Build history of the part. All positions in model axes, mm. Face numbers are marked on the shaded views. A direction names the side the tool comes from. Round coordinates to 2 decimals unless told otherwise and drop trailing zeros. Write each loop counter-clockwise with the first axis right and the second up, starting at its lowest first coordinate (ties: lowest second). Pieces come first, ordered by that corner, then holes. Notation, with made-up numbers: (-9.75, 77) -> (45.25, 77) arc R16 cw to (45.25, 92) -> close; hole circle Ø6 at (70.5, 57.5). An arc over 180 degrees is marked (long way). Return JSON: item names as keys, results as strings.
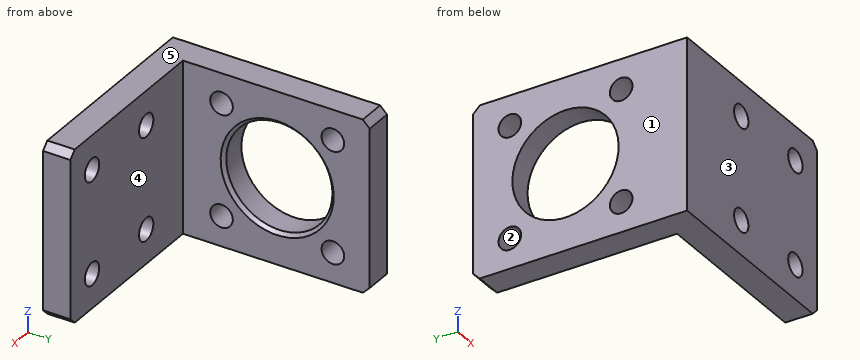
from build123d import *

# Parameters (mm, degrees)
BOSS_EXTRUDE1_DEPTH = 50
HOLE1_D             = 6.6
HOLE2_D             = 31
CHAMFER1_SIZE       = 1
CHAMFER2_SIZE       = 2
HOLE3_D             = 6.6


with BuildPart() as part:
    # Sketch1 → Boss-Extrude1 (new body)
    with BuildSketch(Plane.XY):
        Polygon((-40.819758101, 34.90625), (-40.819758101, -27.59375), (19.180241899, -27.59375), (19.180241899, -19.59375), (-32.819758101, -19.59375), (-32.819758101, 34.90625), align=None)
    extrude(amount=BOSS_EXTRUDE1_DEPTH)

    # Hole1 (through all)
    with Locations(Plane(origin=(-32.819758101, 0, 0), x_dir=(0, 0, -1), z_dir=(1, 0, 0))):
        with Locations((-41.25, 24.15625), (-8.75, 24.15625), (-8.75, -8.34375), (-41.25, -8.34375)):
            Hole(HOLE1_D / 2)

    # Hole2 (through all)
    with Locations(Plane(origin=(-32.819758101, 0, 0), x_dir=(0, 0, -1), z_dir=(1, 0, 0))):
        with Locations((-25, 7.90625)):
            Hole(HOLE2_D / 2)

    # Chamfer1
    chamfer1_edges = [part.edges().sort_by_distance(p)[0] for p in [
        (-32.819758101, 7.90625, 9.5),
    ]]
    chamfer(chamfer1_edges, length=CHAMFER1_SIZE)

    # Chamfer2
    chamfer2_edges = [part.edges().sort_by_distance(p)[0] for p in [
        (19.180241899, -23.59375, 50),
        (-36.819758101, 34.90625, 50),
        (19.180241899, -23.59375, 0),
        (-36.819758101, 34.90625, 0),
    ]]
    chamfer(chamfer2_edges, length=CHAMFER2_SIZE)

    # Hole3 (through all)
    with Locations(Plane(origin=(0, -19.59375, 0), x_dir=(1, 0, 0), z_dir=(0, 1, 0))):
        with Locations((-15.819758101, -40), (-15.819758101, -10), (9.180241899, -10), (9.180241899, -40)):
            Hole(HOLE3_D / 2)


solid = part.part
Q1. Pin check, flat tips, straight feed: pin 1 Ø10.5 at (y, z) = (-8.34, 8.75) entering from +X; pin 2 Ø10.5 at (x, z) = (9.18, 40) entering from +Y. Stop position of each tip, or through.
Verdict:
{"pin 1": "stops at x = -32.82", "pin 2": "stops at y = -19.59"}
Q2. Two-plate mould, pull along Y, no slides. Class the marked faces 1, 2 and 3: +Y half, -Y half, draft (parallel to the pull), parting line (faces both ways), or undercut.
Verdict:
{"face 1": "draft", "face 2": "undercut", "face 3": "-Y half"}
Q3. 3-axis set-ups, long thin cutter, end or side, ignore diameter. For the marked faces 4 and 5: which of +Z, -Z, +X, -X, +Y, -Y reach the whole face in a straight line?
Verdict:
{"face 4": "+Z, -Z, +X, +Y", "face 5": "+Z, +X, -X, +Y, -Y"}
Q4. Saw through at A-A on z = 25. List the corners of the cut face in (x, y).
Verdict:
{"outline": "(-40.82, -27.59) -> (19.18, -27.59) -> (19.18, -19.59) -> (-32.82, -19.59) -> (-32.82, -8.59) -> (-33.82, -7.59) -> (-40.82, -7.59) -> close; (-40.82, 23.41) -> (-33.82, 23.41) -> (-32.82, 24.41) -> (-32.82, 34.91) -> (-40.82, 34.91) -> close"}
Q5. Wall check: L1, parallel to X at y = -22, z = 10; L2, parallel to Y at x = -38, z = 8; L3, parallel to Y at x = 5, z = 7. Give the ranges that are in metal, low to high.
Verdict:
{"L1": "x = -40.82 to -19.12, -12.52 to 5.88, 12.48 to 19.18", "L2": "y = -27.59 to -11.56, -5.13 to 20.94, 27.37 to 34.91", "L3": "y = -27.59 to -19.59"}
Q6. Saw through at B-B on x = -15.5. List the corners of the cut face in (y, z).
Verdict:
{"outline": "(-27.59, 0) -> (-19.59, 0) -> (-19.59, 6.72) -> (-27.59, 6.72) -> close; (-27.59, 13.28) -> (-19.59, 13.28) -> (-19.59, 36.72) -> (-27.59, 36.72) -> close; (-27.59, 43.28) -> (-19.59, 43.28) -> (-19.59, 50) -> (-27.59, 50) -> close"}
Q7. Saw through at C-C on z = 46.5. List the corners of the cut face in (x, y).
Verdict:
{"outline": "(-40.82, -27.59) -> (19.18, -27.59) -> (19.18, -19.59) -> (-32.82, -19.59) -> (-32.82, 34.91) -> (-40.82, 34.91) -> close"}
Q8. Saw through at D-D on x = 5. List the corners of the cut face in (y, z).
Verdict:
{"outline": "(-27.59, 0) -> (-19.59, 0) -> (-19.59, 50) -> (-27.59, 50) -> close"}
